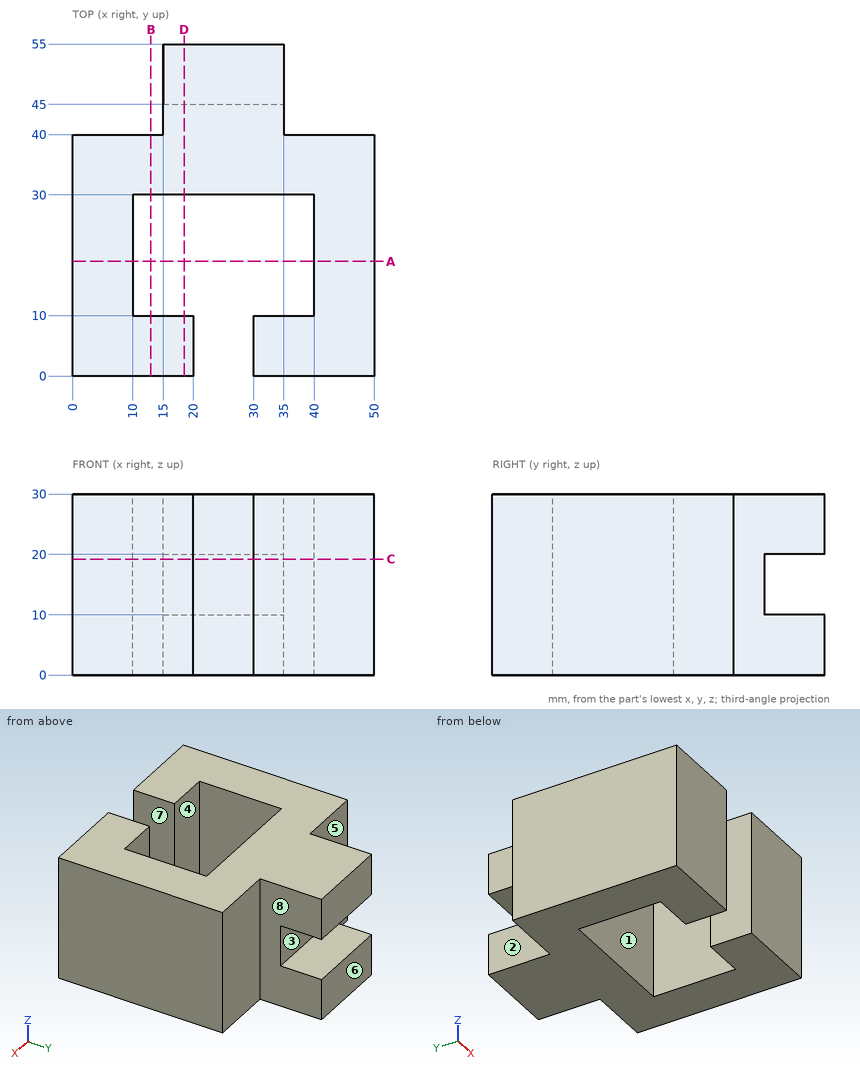
Job drawing, mm, ordinate dimensions from the low corner. One solid piece. A direction names the side the tool comes from. Coordinates: 2 decimals unless noted, no trailing zeros. Order: outer loops, then holes, each group sorted by start corner. A loop starts at its lowest first (then second) coordinate and runs counter-clockwise, first axis right, second up. Notation, with made-up numbers: (-7, 33.25) -> (1, 33.25) arc R15 cw to (1, 58.25) -> close; hole circle Ø6 at (-33.5, 19). An arc over 180 degrees is marked (long way). Return JSON: item names as keys, results as strings. Group by question number.
Item 1: Saw through at B-B on x = 13. Write the cut outline in (y, z).
Item 2: Flat gauge pins, fed straight in: P1, Ø12, axis at x = 8.5, z = 19, coming from the +Y side; P2, Ø6, axis at y = 46, z = 5, coming from the -X side; P3, Ø7.5, axis at y = 48, z = 21, coming from the +X side. Where does each tip first touch, or does it go through?
Item 3: Saw through at D-D on x = 18.5. Write the cut outline in (y, z).
Item 4: Wall check: line 1 along X through (y, z) = (24, 16.5); line 2 along Y through (x, z) = (34, 7.5); line 3 along X through (y, z) = (9, 21.25). Give the ranges that are in metal, low to high. Write a range as [from, to].
Item 5: Pull direction X, two halves, no side cores. Call the marked faces 1, 2 and 3: pulls with the +X half, pulls with the -X half, needs draft (parallel to the pull), parting line crosses it, or undercut.
Item 6: Tool access for the marked faces 4, 5, 6, 7 and 8: list every direction of +Z, -Z, +X, -X, +Y, -Y with a clear straight run to the whole face (end or side of a thin tool).
Item 7: Saw through at C-C on z = 19.25. Write the cut outline in (x, y), then the cut area to 3 significant figures.
Item 8: Saw through at A-A on y = 19. Write the cut outline in (x, z).
Values found:
{
 "1": {"outline": "(0, 0) -> (10, 0) -> (10, 30) -> (0, 30) -> close; (30, 0) -> (40, 0) -> (40, 30) -> (30, 30) -> close"},
 "2": {"P1": "stops at y = 40", "P2": "stops at x = 15", "P3": "stops at x = 35"},
 "3": {"outline": "(0, 0) -> (10, 0) -> (10, 30) -> (0, 30) -> close; (30, 0) -> (55, 0) -> (55, 10) -> (45, 10) -> (45, 20) -> (55, 20) -> (55, 30) -> (30, 30) -> close"},
 "4": {"line 1": "x = [0, 10], [40, 50]", "line 2": "y = [0, 10], [30, 55]", "line 3": "x = [0, 20], [30, 50]"},
 "5": {"face 1": "undercut", "face 2": "pulls with the -X half", "face 3": "needs draft"},
 "6": {"face 4": "+Z, -Z", "face 5": "+Z, -Z, -X, +Y", "face 6": "+Z, -Z, +X, -X, +Y", "face 7": "+Z, -Z, -Y", "face 8": "+Z, -Z, +X, +Y"},
 "7": {"outline": "(0, 0) -> (20, 0) -> (20, 10) -> (10, 10) -> (10, 30) -> (40, 30) -> (40, 10) -> (30, 10) -> (30, 0) -> (50, 0) -> (50, 40) -> (35, 40) -> (35, 45) -> (15, 45) -> (15, 40) -> (0, 40) -> close", "area": "1,400 mm2"},
 "8": {"outline": "(0, 0) -> (10, 0) -> (10, 30) -> (0, 30) -> close; (40, 0) -> (50, 0) -> (50, 30) -> (40, 30) -> close"}
}
